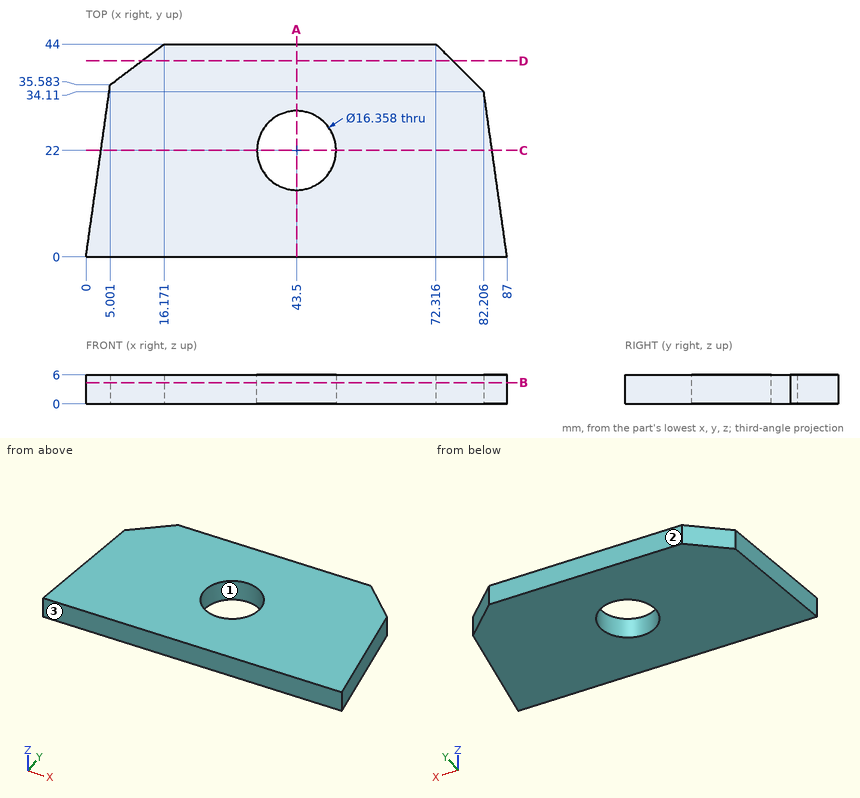
Check sheet for the drawn part. Datum: minimum x, y, z corner. Units: mm. Round coordinates to 2 decimals unless told otherwise and drop trailing zeros. Write each loop counter-clockwise with the first axis right and the second up, starting at its lowest first coordinate (ties: lowest second). Pieces come first, ordered by that corner, then holes. Notation, with made-up numbers: (-23, 78.25) -> (10, 78.25) arc R26 cw to (10, 112.25) -> close; hole circle Ø6 at (-24, 59.25). An arc over 180 degrees is marked (long way). Put each result on its own line as item: value.
(1) Go/stop test with flat-tipped pins: pin 1 Ø3 at (y, z) = (13.5, 4) entering from -X; pin 2 Ø1.5 at (y, z) = (6, 3) entering from -X. Record where each tip stops, or that it passes through.
Values found:
pin 1: stops at x = 1.69
pin 2: stops at x = 0.74
(2) Sectioned sample at D-D (y = 40.5). Enter the section's corners in (x, z), plus the area to 3 significant figures.
Values found:
outline: (11.53, 0) -> (75.82, 0) -> (75.82, 6) -> (11.53, 6) -> close
area: 386 mm^2
(3) Sectioned sample at A-A (x = 43.5). Enter the section's corners in (y, z), plus the area to 3 significant figures.
Values found:
outline: (0, 0) -> (13.82, 0) -> (13.82, 6) -> (0, 6) -> close; (30.18, 0) -> (44, 0) -> (44, 6) -> (30.18, 6) -> close
area: 166 mm^2
(4) Sectioned sample at B-B (z = 4.4). Enter the section's corners in (x, y).
Values found:
outline: (0, 0) -> (87, 0) -> (82.21, 34.11) -> (72.32, 44) -> (16.17, 44) -> (5, 35.58) -> close; hole circle Ø16.36 at (43.5, 22)
(5) Sectioned sample at C-C (y = 22). Enter the section's corners in (x, z).
Values found:
outline: (3.09, 0) -> (35.32, 0) -> (35.32, 6) -> (3.09, 6) -> close; (51.68, 0) -> (83.91, 0) -> (83.91, 6) -> (51.68, 6) -> close
(6) Material ranges on line 1 (Y direction, x = 43.5, z = 2); line 2 (Y direction, x = 39, z = 2.3); line 3 (X direction, y = 25.5, z = 3.15) (1 decimal), recorded low to high.
Values found:
line 1: y = 0 to 13.82, 30.18 to 44
line 2: y = 0 to 15.17, 28.83 to 44
line 3: x = 3.6 to 36.1, 50.9 to 83.4
(7) Mould release check, pull along Y, two halves, no side actions. Record for the marked faces 1, 2 and 3: released by +Y, released by -Y, zero draft, split by the parting line, or undercut.
Values found:
face 1: undercut
face 2: released by +Y
face 3: released by -Y
